Can you work these out from the model? Positions are in its coordinate system, mm. A direction names the side the tool comes from. Coordinates: 2 decimals unless noted, no trailing zeros. Order: outer loops, then holes, each group sorted by start corner. A loop starts at its lowest first (then second) coordinate and runs counter-clockwise, first axis right, second up. Notation, with made-up numbers: (33.25, 75.5) - (40.25, 75.5) arc R9 ccw to (40.25, 87.5) - close; hole circle Ø6 at (-21.75, 47). An arc over 180 degrees is marked (long way). Use a Markdown table: item, result. Add a question column.
(1) On a 3-axis mill with a long thin cutter (end or side, diameter ignored), from which of +Z, -Z, +X, -X, +Y, -Y can I reach the whole of each face in a straight line? I mean faces 1 (the flat face through (-12, 60, 20)), 2 (the cylindrical face through (-63.763, -36.302, 10.874)). Say none if no direction works.
(2) If I drill on L1, parallel to Y at x = 0, z = 9.5; L2, parallel to Y at x = -63, z = 13.5; L3, parallel to X at y = 35, z = 13.5, over which ranges is the centre line in solid material (lowest first)? Write a range as [from, to].
(3) I want a section at D-D (x = 69). List the corners of the cut face in (y, z) for me.
(4) I want a section at B-B (x = 38.5). List the corners of the cut face in (y, z) for me.
(5) I want a section at C-C (z = 7.75). List the corners of the cut face in (x, y) for me.
(6) I want a section at A-A (y = 0). List the corners of the cut face in (x, z) for me, and give its area (3 significant figures).
(7) For pin 1 Ø10 at (y, z) = (-42, 14.5) entering from -X; pin 2 Ø1 at (y, z) = (1, 2) entering from -X; pin 3 Ø1 at (y, z) = (30, 2.5) entering from -X, each with a flat end and sliding along its axis, tell me the tip position at first contact or that it passes through.
(8) We'd pull the mould along X, two halves only. Please class faces 3 (the flat face through (11, 60, 0)), 4 (the cylindrical face through (64.02, 35.15, 10.87)), 5 (the conical face through (-60.706, 35.644, 0.347)), 6 (the cylindrical face through (-17.34, -78.1, 9.86)): pulls with the +X half, pulls with the -X half, needs draft (parallel to the pull), parting line crosses it, or undercut.
```python
from build123d import *

# Parameters (mm, degrees)
SKETCH1_R             = 80
SKETCH1_R_2           = 60
BOSS_EXTRUDE1_DEPTH   = 20
M8_TAPPED_HOLE1_D     = 6.8
M8_TAPPED_HOLE1_DEPTH = 18
M8_TAPPED_HOLE1_TIP   = 2.042926105


with BuildPart() as part:
    # Sketch1 → Boss-Extrude1 (new body)
    with BuildSketch(Plane.XY):
        Circle(SKETCH1_R)
        Circle(SKETCH1_R_2, mode=Mode.SUBTRACT)
    extrude(amount=BOSS_EXTRUDE1_DEPTH)

    # M8 Tapped Hole1
    with Locations(Plane(origin=(0, 70, 20), x_dir=(1, 0, 0), z_dir=(0, 0, 1))):
        with Locations((0, 0), (60.621778265, -35), (60.621778265, -105), (0, -140), (-60.621778265, -105), (-60.621778265, -35)):
            Hole(M8_TAPPED_HOLE1_D / 2, depth=M8_TAPPED_HOLE1_DEPTH)
            with Locations((0, 0, -(M8_TAPPED_HOLE1_DEPTH + M8_TAPPED_HOLE1_TIP / 2))):  # 118° drill point
                Cone(0, M8_TAPPED_HOLE1_D / 2, M8_TAPPED_HOLE1_TIP, mode=Mode.SUBTRACT)


solid = part.part
```
Answers follow:
| question | item | result |
|---|---|---|
| 1 | face 1 | +Z, +X, -X, +Y, -Y |
| 1 | face 2 | +Z |
| 2 | L1 | y = [-80, -73.4], [-66.6, -60], [60, 66.6], [73.4, 80] |
| 2 | L2 | y = [-49.31, -37.43], [-32.57, 32.57], [37.43, 49.31] |
| 2 | L3 | x = [-71.94, -64.02], [-57.22, -48.73], [48.73, 57.22], [64.02, 71.94] |
| 3 | outline | (-40.48, 0) - (40.48, 0) - (40.48, 20) - (-40.48, 20) - close |
| 4 | outline | (-70.13, 0) - (-46.02, 0) - (-46.02, 20) - (-70.13, 20) - close; (46.02, 0) - (70.13, 0) - (70.13, 20) - (46.02, 20) - close |
| 5 | outline | circle Ø160 at (0, 0); hole circle Ø6.8 at (-60.62, -35); hole circle Ø6.8 at (-60.62, 35); hole circle Ø120 at (0, 0); hole circle Ø6.8 at (0, -70); hole circle Ø6.8 at (0, 70); hole circle Ø6.8 at (60.62, -35); hole circle Ø6.8 at (60.62, 35) |
| 6 | outline | (-80, 0) - (-60, 0) - (-60, 20) - (-80, 20) - close; (60, 0) - (80, 0) - (80, 20) - (60, 20) - close |
| 6 | area | 800 mm² |
| 7 | pin 1 | stops at x = -70.93 |
| 7 | pin 2 | stops at x = -80 |
| 7 | pin 3 | stops at x = -74.36 |
| 8 | face 3 | needs draft |
| 8 | face 4 | undercut |
| 8 | face 5 | undercut |
| 8 | face 6 | parting line crosses it |
